Can you work these out from the drawing? Everything is in mm from the part's minimum corner. A direction names the side the tool comes from. Give positions to 0.01 mm unless a question says otherwise; leave off trailing zeros. Order: outer loops, then holes, each group sorted by start corner. A loop starts at its lowest first (then second) coordinate and runs counter-clockwise, first axis right, second up. Notation, with made-up numbers: (24.5, -10) - (48.5, -10) arc R27 ccw to (48.5, 10) - close; hole circle Ø3 at (14, -31.75). An arc over 180 degrees is marked (long way). Answer as a JSON object with one key per item and string values.
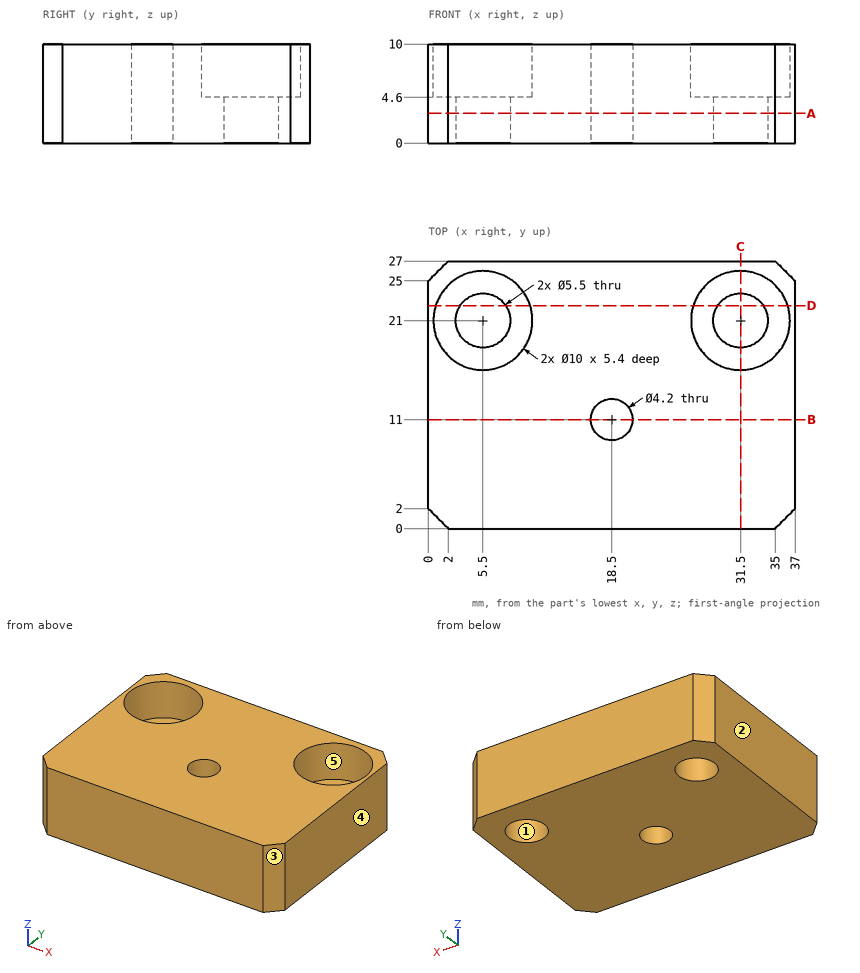
Q1. If we section it at C-C, the plane x = 31.5: Please give me the cut outline in (y, z), then the cut area to 3 significant figures.
Recorded:
{"outline": "(0, 0) - (18.25, 0) - (18.25, 4.6) - (16, 4.6) - (16, 10) - (0, 10) - close; (23.75, 0) - (27, 0) - (27, 10) - (26, 10) - (26, 4.6) - (23.75, 4.6) - close", "area": "191 mm^2"}
Q2. I need wall thicknesses on L1, parallel to Y at x = 31.5, z = 1.6; L2, parallel to X at y = 20, z = 7.5; L3, parallel to Y at x = 18.5, z = 3.75. Which ranges of each line are inside material? Lowest first, please.
Recorded:
{"L1": "y = 0 to 18.25, 23.75 to 27", "L2": "x = 0 to 0.6, 10.4 to 26.6, 36.4 to 37", "L3": "y = 0 to 8.9, 13.1 to 27"}
Q3. Which directions (+Z, -Z, +X, -X, +Y, -Y) give clear straight access to the entire face, cutting with the end or side of a thin tool? Please do the marked faces 4 and 5.
Recorded:
{"face 4": "+Z, -Z, +X, +Y, -Y", "face 5": "+Z"}
Q4. If we section it at B-B, the plane y = 11: Please give me the cut outline in (x, z), then the cut area to 3 significant figures.
Recorded:
{"outline": "(0, 0) - (16.4, 0) - (16.4, 10) - (0, 10) - close; (20.6, 0) - (37, 0) - (37, 10) - (20.6, 10) - close", "area": "328 mm^2"}
Q5. I'm going to push flat-ended pins straight in: pin 1 Ø5 at (x, y) = (31.5, 21) entering from +Z; pin 2 Ø6 at (x, y) = (5.5, 21) entering from +Z. Where does each tip first touch, or does it pass through?
Recorded:
{"pin 1": "passes through", "pin 2": "stops at z = 4.6"}
Q6. If we section it at D-D, the plane y = 22.5: Please give me the cut outline in (x, z).
Recorded:
{"outline": "(0, 0) - (3.2, 0) - (3.2, 4.6) - (0.73, 4.6) - (0.73, 10) - (0, 10) - close; (7.8, 0) - (29.2, 0) - (29.2, 4.6) - (26.73, 4.6) - (26.73, 10) - (10.27, 10) - (10.27, 4.6) - (7.8, 4.6) - close; (33.8, 0) - (37, 0) - (37, 10) - (36.27, 10) - (36.27, 4.6) - (33.8, 4.6) - close"}
Q7. We'd pull the mould along X, two halves only. Please class the marked faces 1, 2 and 3: released by +X, released by -X, zero draft, split by the parting line, or undercut.
Recorded:
{"face 1": "undercut", "face 2": "released by -X", "face 3": "released by +X"}
Q8. If we section it at A-A, the plane z = 3: Please give me the cut outline in (x, y), then the cut area to 3 significant figures.
Recorded:
{"outline": "(0, 2) - (2, 0) - (35, 0) - (37, 2) - (37, 25) - (35, 27) - (2, 27) - (0, 25) - close; hole circle Ø5.5 at (5.5, 21); hole circle Ø4.2 at (18.5, 11); hole circle Ø5.5 at (31.5, 21)", "area": "930 mm^2"}
